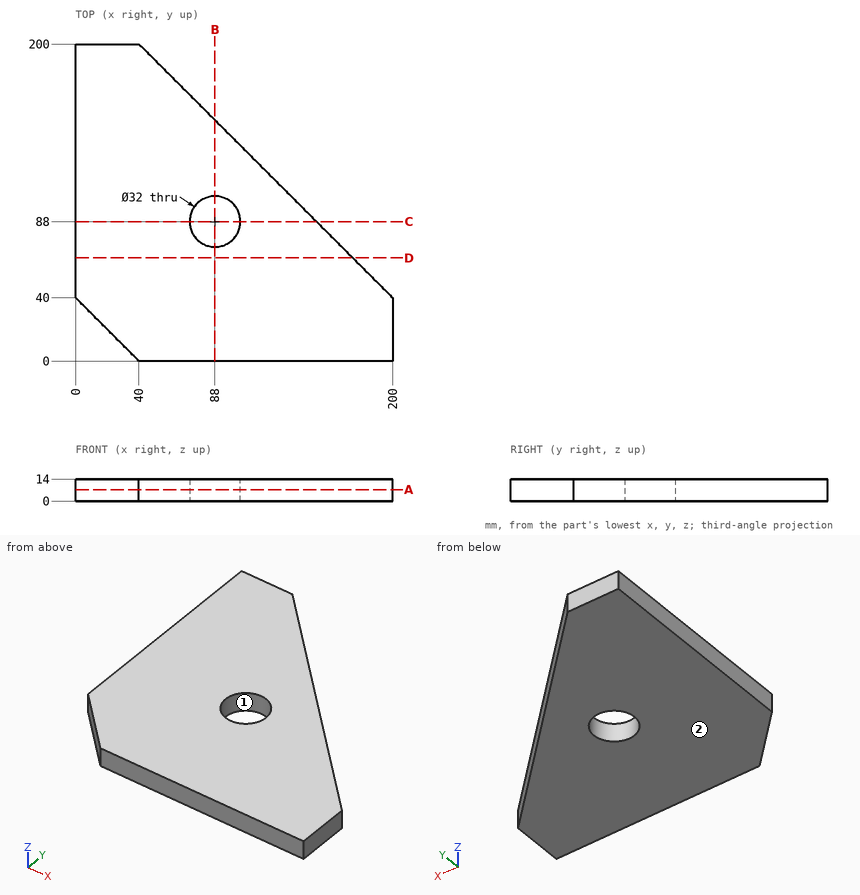
Study the drawing (mm; zero at the part's minimum x, y, z) and answer. Give positions to 0.01 mm unless a question says otherwise; leave off trailing zeros. Write each loop counter-clockwise with the first axis right and the second up, starting at its lowest first coordinate (ties: lowest second). Pieces come first, ordered by that corner, then holes.
Item 1: Section B-B, the plane x = 88 is taken. Write down the section's boundary in (y, z).
Item 2: Find the intervals of material crossed by line 1 along Y through (x, z) = (136, 7); line 2 along X through (y, z) = (92.5, 9.5); line 3 along Y through (x, z) = (88, 5.75), in increasing order.
Item 3: Determine the mould class of the marked faces 1 and 2 for opening direction Y: released by +Y, released by -Y, zero draft, split by the parting line, or undercut.
Item 4: Section D-D, the plane y = 65 is taken. Write down the section's boundary in (x, z).
Item 5: A flat-ended cylindrical pin translates along its axis: P1, Ø1.5, axis at x = 131.5, z = 12, coming from the +Y side. Find the tip coordinate at first contact, or state that the pin passes through.
Item 6: Section A-A, the plane z = 7.25 is taken. Write down the section's boundary in (x, y).
Completed:
1. outline: (0, 0) - (72, 0) - (72, 14) - (0, 14) - close; (104, 0) - (152, 0) - (152, 14) - (104, 14) - close
2. line 1: y = 0 to 104
2. line 2: x = 0 to 72.65, 103.35 to 147.5
2. line 3: y = 0 to 72, 104 to 152
3. face 1: undercut
3. face 2: zero draft
4. outline: (0, 0) - (175, 0) - (175, 14) - (0, 14) - close
5. P1: stops at y = 109.25
6. outline: (0, 40) - (40, 0) - (200, 0) - (200, 40) - (40, 200) - (0, 200) - close; hole circle Ø32 at (88, 88)
